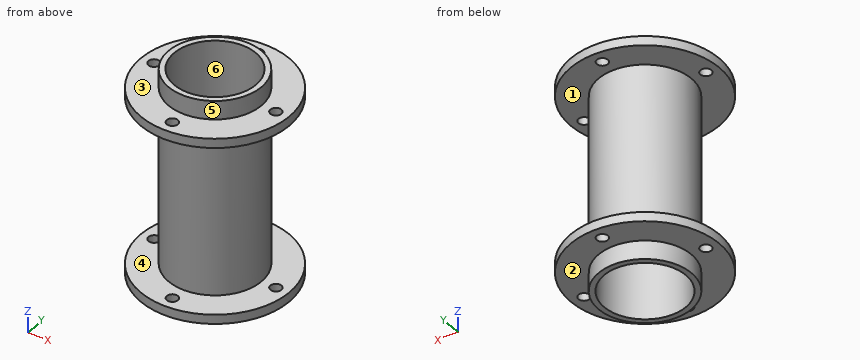
```python
from build123d import *

# Parameters (mm, degrees)
SKETCH1_R           = 25
SKETCH1_R_2         = 22
BOSS_EXTRUDE1_DEPTH = 60
BOSS_EXTRUDE2_START = -15
SKETCH2_R           = 40
SKETCH2_R_2         = 25
SKETCH2_R_3         = 3
BOSS_EXTRUDE2_DEPTH = 5


with BuildPart() as part:
    # Sketch1 → Boss-Extrude1 (new, symmetric)
    with BuildSketch(Plane.XY):
        Circle(SKETCH1_R)
        Circle(SKETCH1_R_2, mode=Mode.SUBTRACT)
    extrude(amount=BOSS_EXTRUDE1_DEPTH, both=True)

    # Sketch2 → Boss-Extrude2 (add)
    with BuildSketch(Plane(origin=(0, 0, -60), x_dir=(-1, 0, 0), z_dir=(0, 0, -1)).offset(BOSS_EXTRUDE2_START)):
        Circle(SKETCH2_R)
        Circle(SKETCH2_R_2, mode=Mode.SUBTRACT)
        with Locations((0, 33)):
            Circle(SKETCH2_R_3, mode=Mode.SUBTRACT)
        with Locations((33, 0)):
            Circle(SKETCH2_R_3, mode=Mode.SUBTRACT)
        with Locations((0, -33)):
            Circle(SKETCH2_R_3, mode=Mode.SUBTRACT)
        with Locations((-33, 0)):
            Circle(SKETCH2_R_3, mode=Mode.SUBTRACT)
    boss_extrude2 = extrude(amount=BOSS_EXTRUDE2_DEPTH)

    # Mirror1: Boss-Extrude2 across plane
    add(boss_extrude2.mirror(Plane.XY))


solid = part.part
```
Can you work these out from the model? Positions are in its coordinate system, mm. Face numbers are marked on the shaded views. A direction names the side the tool comes from. Coordinates: 2 decimals unless noted, no trailing zeros. Order: outer loops, then holes, each group sorted by start corner. A loop starts at its lowest first (then second) coordinate and runs counter-clockwise, first axis right, second up. Notation, with made-up numbers: (16, -14) - (60, -14) arc R6 cw to (60, -5) - close; hole circle Ø7 at (45, -35). An arc over 180 degrees is marked (long way). Answer in a Markdown table with one row per item.
1. Suppose I cut it at A-A (x = -15). Please give me the cut outline in (y, z), and give its area (3 significant figures).
Reply:
| item | result |
|---|---|
| outline | (-37.08, -50) - (-20, -50) - (-20, -60) - (-16.09, -60) - (-16.09, 60) - (-20, 60) - (-20, 50) - (-37.08, 50) - (-37.08, 45) - (-20, 45) - (-20, -45) - (-37.08, -45) - close; (16.09, -60) - (20, -60) - (20, -50) - (37.08, -50) - (37.08, -45) - (20, -45) - (20, 45) - (37.08, 45) - (37.08, 50) - (20, 50) - (20, 60) - (16.09, 60) - close |
| area | 1,280 mm^2 |
2. If we mould it in two halves opening along Y, with no side actions, what happens to the marked faces 4, 5 and 6? For each: pulls with the +Y half, pulls with the -Y half, needs draft (parallel to the pull), parting line crosses it, or undercut.
Reply:
| item | result |
|---|---|
| face 4 | needs draft |
| face 5 | parting line crosses it |
| face 6 | undercut |
3. Suppose I cut it at C-C (x = 34.5). Please give me the cut outline in (y, z), and give its area (3 significant figures).
Reply:
| item | result |
|---|---|
| outline | (-20.24, -50) - (-2.6, -50) - (-2.6, -45) - (-20.24, -45) - close; (-20.24, 45) - (-2.6, 45) - (-2.6, 50) - (-20.24, 50) - close; (2.6, -50) - (20.24, -50) - (20.24, -45) - (2.6, -45) - close; (2.6, 45) - (20.24, 45) - (20.24, 50) - (2.6, 50) - close |
| area | 353 mm^2 |
4. Suppose I cut it at D-D (z = 52.5). Please give me the cut outline in (x, y), and give its area (3 significant figures).
Reply:
| item | result |
|---|---|
| outline | circle Ø50 at (0, 0); hole circle Ø44 at (0, 0) |
| area | 443 mm^2 |
5. For pin 1 (7 mm diameter, centred on x = -33, y = 0, fed in from +Z); pin 2 (10 mm diameter, centred on x = 24, y = -32, fed in from -Z); pin 3 (5 mm diameter, centred on x = -3.5, z = 10, fed in from -Y), each with a flat end and sliding along its axis, tell me the tip position at first contact or that it passes through.
Reply:
| item | result |
|---|---|
| pin 1 | stops at z = 50 |
| pin 2 | stops at z = -50 |
| pin 3 | stops at y = -24.98 |
6. Suppose I cut it at B-B (y = -6). Please give me the cut outline in (x, z), and give its area (3 significant figures).
Reply:
| item | result |
|---|---|
| outline | (-39.55, -50) - (-24.27, -50) - (-24.27, -60) - (-21.17, -60) - (-21.17, 60) - (-24.27, 60) - (-24.27, 50) - (-39.55, 50) - (-39.55, 45) - (-24.27, 45) - (-24.27, -45) - (-39.55, -45) - close; (21.17, -60) - (24.27, -60) - (24.27, -50) - (39.55, -50) - (39.55, -45) - (24.27, -45) - (24.27, 45) - (39.55, 45) - (39.55, 50) - (24.27, 50) - (24.27, 60) - (21.17, 60) - close |
| area | 1,050 mm^2 |
7. For the marked faces 1, 2 and 3, which set-ups out of +Z, -Z, +X, -X, +Y, -Y let a thin tool reach every point of the face, with its end or its side?
Reply:
| item | result |
|---|---|
| face 1 | none |
| face 2 | -Z |
| face 3 | +Z |
8. If I drill on line 1 along Y through (x, z) = (0, 47); line 2 along Z through (x, y) = (31.5, -13); line 3 along X through (y, z) = (1, 31), over which ranges is the centre line in solid material (lowest first)?
Reply:
| item | result |
|---|---|
| line 1 | y = -40 to -36, -30 to -22, 22 to 30, 36 to 40 |
| line 2 | z = -50 to -45, 45 to 50 |
| line 3 | x = -24.98 to -21.98, 21.98 to 24.98 |
